```python
from build123d import *

# Parameters (mm, degrees)
SKETCH_1_W      = 60
SKETCH_1_H      = 60
SKETCH_1_R      = 20
EXTRUDE_1_DEPTH = 10
CHAMFER_1_SIZE  = 10
CHAMFER_3_SIZE  = 2


with BuildPart() as part:
    # 草图1 → 凸台-拉伸1 (new body)
    with BuildSketch(Plane.XY):
        Rectangle(SKETCH_1_W, SKETCH_1_H)
        Circle(SKETCH_1_R, mode=Mode.SUBTRACT)
    extrude(amount=EXTRUDE_1_DEPTH)

    # 倒角1
    chamfer_1_edges = [part.edges().sort_by_distance(p)[0] for p in [
        (30, -30, 5),
        (-30, -30, 5),
    ]]
    chamfer(chamfer_1_edges, length=CHAMFER_1_SIZE)

    # 倒角3
    chamfer_3_edges = [part.edges().sort_by_distance(p)[0] for p in [
        (-20, 0, 0),
        (-20, 0, 10),
    ]]
    chamfer(chamfer_3_edges, length=CHAMFER_3_SIZE)


solid = part.part
```
Geometry check sheet. Reference: the model listing, model coordinates, mm. Give positions to 0.01 mm unless a question says otherwise; leave off trailing zeros. Write each loop counter-clockwise with the first axis right and the second up, starting at its lowest first coordinate (ties: lowest second). Pieces come first, ordered by that corner, then holes.
1) Release check for a two-part mould opening along Y. For faces 1 (the flat face through (30, 5, 5)), 2 (the flat face through (0, -30, 5)), 3 (the cylindrical face through (-4.336, -19.524, 4.958)) record: pulls with the +Y half, pulls with the -Y half, needs draft (parallel to the pull), parting line crosses it, or undercut.
2) Gauge pin test, flat end, axial feed: pin 1 (4 mm diameter, centred on x = 20.5, z = 8, fed in from -Y). Record the tip position at first contact, or that the pin passes through.
3) Section check A-A, the plane x = 0. Record the boundary of the cut face in (y, z).
4) Section check B-B, the plane z = 7.25. Record the boundary of the cut face in (x, y).
5) Material ranges on L1, parallel to Y at x = 0, z = 6.25; L2, parallel to Y at x = 7, z = 9; L3, parallel to X at y = -17, z = 7.75, recorded low to high.
6) Section check D-D, the plane y = -26. Record the boundary of the cut face in (x, z).
Computed:
1. face 1: needs draft
1. face 2: pulls with the -Y half
1. face 3: undercut
2. pin 1: stops at y = -30
3. outline: (-30, 0) - (-22, 0) - (-20, 2) - (-20, 8) - (-22, 10) - (-30, 10) - close; (20, 2) - (22, 0) - (30, 0) - (30, 10) - (22, 10) - (20, 8) - close
4. outline: (-30, -20) - (-20, -30) - (20, -30) - (30, -20) - (30, 30) - (-30, 30) - close; hole circle Ø40 at (0, 0)
5. L1: y = -30 to -20, 20 to 30
5. L2: y = -30 to -19.8, 19.8 to 30
5. L3: x = -30 to -10.54, 10.54 to 30
6. outline: (-24, 0) - (24, 0) - (24, 10) - (-24, 10) - close
